from build123d import *

# Parameters (mm, degrees)
SHANK_END_CHAMFER_6X45_SIZE = 6


with BuildPart() as part:
    # Pin Profile Sketch → Pin Body Revolve (revolve)
    with BuildSketch(Plane.XY, mode=Mode.PRIVATE) as pin_body_revolve_sk:
        Polygon((50, 0), (50, 250), (75, 250), (75, 300), (31.5, 300), (31.5, 0), align=None)
    revolve(pin_body_revolve_sk.sketch.rotate(Axis((0, 0, 0), (0, 1, 0)), 90), axis=Axis((0, 0, 0), (0, 1, 0)))

    # Shank End Chamfer 6x45°
    shank_end_chamfer_6x45_edges = [part.edges().sort_by_distance(p)[0] for p in [
        (0, 0, 50),
    ]]
    chamfer(shank_end_chamfer_6x45_edges, length=SHANK_END_CHAMFER_6X45_SIZE)


solid = part.part
Check sheet for the modelled part. Datum: model origin and axes. Units: mm. Coordinates: 2 decimals unless noted, no trailing zeros. Loops run counter-clockwise (first coordinate to the right, second up) from the corner with the lowest first, then second, coordinate; pieces in that order, holes last. Notation, with made-up numbers: (43, 62) -> (67, 62) arc R14 cw to (67, 77) -> close; hole circle Ø3 at (73, 0). An arc over 180 degrees is marked (long way). Write item = value, one per line. Start each with the question number.
1. Section check A-A on x = 0. Record the cut outline in (y, z), then the cut area to 3 significant figures.
2. Draft check along Z on faces 1 (the cylindrical face through (-15.02, 129.71, -47.69)), 2 (the cylindrical face through (-31.232, 147.9, 4.101)), 3 (the flat face through (16, 250, 49)). Enter one of: released by +Z, released by -Z, zero draft, split by the parting line, or undercut.
3. Section check C-C on y = 69. Record the cut outline in (x, z), then the cut area to 3 significant figures.
4. Section check B-B on z = 0. Record the cut outline in (x, y), then the cut area to 3 significant figures.
5. Material ranges on line 1 (Z direction, x = -1.5, y = 97.5); line 2 (X direction, y = 210.5, z = 0); line 3 (Y direction, x = -47, z = -49), recorded low to high.
6. Section check D-D on y = 278.5. Record the cut outline in (x, z), then the cut area to 3 significant figures.
7. Depth check by flat-ended pin: P1, Ø1, axis at x = 20.5, z = 60, coming from the -Y side; P2, Ø8, axis at x = 28.5, y = 181.5, coming from the +Z side; P3, Ø10, axis at x = -0.5, y = 152.5, coming from the +Z side. Enter the tip coordinate at first touch or a pass-through.
Responses:
q1.outline = (0, -44) -> (6, -50) -> (250, -50) -> (250, -75) -> (300, -75) -> (300, -31.5) -> (0, -31.5) -> close; (0, 31.5) -> (300, 31.5) -> (300, 75) -> (250, 75) -> (250, 50) -> (6, 50) -> (0, 44) -> close
q1.area = 13,600 mm2
q2.face_1 = split by the parting line
q2.face_2 = undercut
q2.face_3 = zero draft
q3.outline = circle Ø100 at (0, 0); hole circle Ø63 at (0, 0)
q3.area = 4,740 mm2
q4.outline = (-75, 250) -> (-50, 250) -> (-50, 6) -> (-44, 0) -> (-31.5, 0) -> (-31.5, 300) -> (-75, 300) -> close; (31.5, 0) -> (44, 0) -> (50, 6) -> (50, 250) -> (75, 250) -> (75, 300) -> (31.5, 300) -> close
q4.area = 13,600 mm2
q5.line_1 = -49.98 to -31.46, 31.46 to 49.98
q5.line_2 = -50 to -31.5, 31.5 to 50
q5.line_3 = 250 to 300
q6.outline = circle Ø150 at (0, 0); hole circle Ø63 at (0, 0)
q6.area = 14,600 mm2
q7.P1 = 250
q7.P2 = 43.59
q7.P3 = 50
